Part model, mm, in its own coordinate system. Face numbers are marked on the shaded views. Round coordinates to 2 decimals unless told otherwise and drop trailing zeros. Write each loop counter-clockwise with the first axis right and the second up, starting at its lowest first coordinate (ties: lowest second). Pieces come first, ordered by that corner, then holes. Notation, with made-up numbers: M 73,75 L 94,75 A30 cw 94,107 Z; hole C -19.75,75 d7. An arc over 180 degrees is marked long. Use a Markdown table: item, result. Add a question column.
1) Two-plate mould, pull along X, no slides. Class the marked faces 1, 2, 3 and 4: released by +X, released by -X, zero draft, split by the parting line, or undercut.
2) Slice it at B-B on z = 0. Write the cut outline in (x, y).
3) Wall check: probe 1 along X at (y, z) = (0.5, 0.25); probe 2 along X at (y, z) = (3.25, 1.25); probe 3 along Z at (x, y) = (-10, -2). Give the ranges that are in metal, low to high.
4) Slice it at D-D on x = -3. Write the cut outline in (y, z).
5) Slice it at C-C on y = -5. Write the cut outline in (x, z), plus the area to 3 significant figures.
6) Slice it at A-A on x = 13. Write the cut outline in (y, z), plus the area to 3 significant figures.
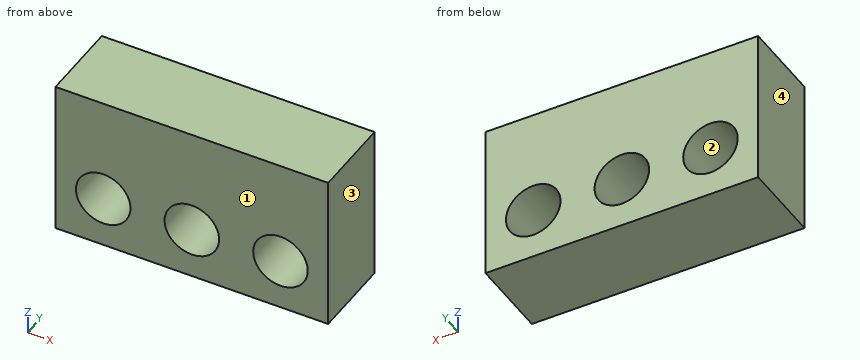
```python
from build123d import *

# Parameters (mm, degrees)
SKETCH_1_W          = 40
SKETCH_1_H          = 12
EXTRUDE_1_DEPTH     = 7.5
CUT_EXTRUDE_1_REACH = 26.5
SKETCH_2_R          = 4
CUT_EXTRUDE_2_REACH = 26.5
SKETCH_3_R          = 4
SKETCH_6_W          = 40
SKETCH_6_H          = 12
EXTRUDE_3_DEPTH     = 8


with BuildPart() as part:
    # 草图1 → 凸台-拉伸1 (new, symmetric)
    with BuildSketch(Plane.XY):
        Rectangle(SKETCH_1_W, SKETCH_1_H)
    extrude(amount=EXTRUDE_1_DEPTH, both=True)

    # 草图2 → 切除-拉伸1 (cut, up to next)
    with BuildSketch(Plane(origin=(0, 6, 0), x_dir=(1, 0, 0), z_dir=(0, 1, 0)), mode=Mode.PRIVATE) as cut_extrude_1_sk1:
        with Locations(Location((-13, 0, 0), (0, 0, 270))):
            Circle(SKETCH_2_R)
    cut_extrude_1_tool1 = extrude(cut_extrude_1_sk1.sketch, amount=-CUT_EXTRUDE_1_REACH, mode=Mode.PRIVATE) & part.part
    # 草图2 → 切除-拉伸1 (cut, up to next)
    with BuildSketch(Plane(origin=(0, 6, 0), x_dir=(1, 0, 0), z_dir=(0, 1, 0)), mode=Mode.PRIVATE) as cut_extrude_1_sk2:
        with Locations(Location((13, 0, 0), (0, 0, 270))):
            Circle(SKETCH_2_R)
    cut_extrude_1_tool2 = extrude(cut_extrude_1_sk2.sketch, amount=-CUT_EXTRUDE_1_REACH, mode=Mode.PRIVATE) & part.part
    add(cut_extrude_1_tool1.solids().sort_by_distance((-13, 6, 0))[0], mode=Mode.SUBTRACT)
    add(cut_extrude_1_tool2.solids().sort_by_distance((13, 6, 0))[0], mode=Mode.SUBTRACT)

    # 草图3 → 切除-拉伸2 (cut, up to next)
    with BuildSketch(Plane.XZ.offset(6), mode=Mode.PRIVATE) as cut_extrude_2_sk1:
        with Locations(Location((0, 0, 0), (0, 0, 270))):
            Circle(SKETCH_3_R)
    cut_extrude_2_tool1 = extrude(cut_extrude_2_sk1.sketch, amount=-CUT_EXTRUDE_2_REACH, mode=Mode.PRIVATE) & part.part
    add(cut_extrude_2_tool1.solids().sort_by_distance((0, -6, 0))[0], mode=Mode.SUBTRACT)

    # 草图6 → 凸台-拉伸3 (add)
    with BuildSketch(Plane.XY.offset(7.5)):
        Rectangle(SKETCH_6_W, SKETCH_6_H)
    extrude(amount=EXTRUDE_3_DEPTH)


solid = part.part
```
Entries:
| question | item | result |
|---|---|---|
| 1 | face 1 | zero draft |
| 1 | face 2 | undercut |
| 1 | face 3 | released by +X |
| 1 | face 4 | released by -X |
| 2 | outline | M -20,-6 L -17,-6 L -17,6 L -20,6 Z; M -9,-6 L -4,-6 L -4,6 L -9,6 Z; M 4,-6 L 9,-6 L 9,6 L 4,6 Z; M 17,-6 L 20,-6 L 20,6 L 17,6 Z |
| 3 | probe 1 | x = -20 to -16.99, -9.01 to -3.99, 3.99 to 9.01, 16.99 to 20 |
| 3 | probe 2 | x = -20 to -16.8, -9.2 to -3.8, 3.8 to 9.2, 16.8 to 20 |
| 3 | probe 3 | z = -7.5 to -2.65, 2.65 to 15.5 |
| 4 | outline | M -6,-7.5 L 6,-7.5 L 6,-2.65 L -6,-2.65 Z; M -6,2.65 L 6,2.65 L 6,15.5 L -6,15.5 Z |
| 5 | outline | M -20,-7.5 L 20,-7.5 L 20,15.5 L -20,15.5 Z; hole C -13,0 d8; hole C 0,0 d8; hole C 13,0 d8 |
| 5 | area | 769 mm^2 |
| 6 | outline | M -6,-7.5 L 6,-7.5 L 6,-4 L -6,-4 Z; M -6,4 L 6,4 L 6,15.5 L -6,15.5 Z |
| 6 | area | 180 mm^2 |
